from build123d import *

# Parameters (mm, degrees)
SKETCH_2_R          = 6
CUT_EXTRUDE_1_DEPTH = 8
SKETCH_3_W          = 2.5
SKETCH_3_H          = 3
SKETCH_4_W          = 1.25
SKETCH_4_H          = 32


with BuildPart() as part:
    # 草图1 → 旋转1 (revolve)
    with BuildSketch(Plane.XY, mode=Mode.PRIVATE) as revolve_1_sk:
        Polygon((0, 41), (3, 41), (5, 40.647346039), (5, 33.535898385), (3, 33), (3.3865, 33), (4, 32.3865), (4, 18.6135), (3.3865, 18), (2.45, 18), (2.45, 12), (0, 12), align=None)
    revolve(revolve_1_sk.sketch.rotate(Axis((0, 12, 0), (0, 1, 0)), 180), axis=Axis((0, 12, 0), (0, 1, 0)))

    # 草图2 → 切除-拉伸1 (cut)
    with BuildSketch(Plane(origin=(0, 33, 0), x_dir=(1, 0, 0), z_dir=(0, 1, 0))):
        Circle(SKETCH_2_R)
        Polygon((-3.464101615, 0), (-1.732050808, -3), (1.732050808, -3), (3.464101615, 0), (1.732050808, 3), (-1.732050808, 3), align=None, mode=Mode.SUBTRACT)
    extrude(amount=CUT_EXTRUDE_1_DEPTH, mode=Mode.SUBTRACT)

    # 草图3 → 旋转2 (revolve)
    with BuildSketch(Plane.XY, mode=Mode.PRIVATE) as revolve_2_sk:
        with Locations((1.25, 42.5)):
            Rectangle(SKETCH_3_W, SKETCH_3_H)
    revolve(revolve_2_sk.sketch.rotate(Axis((0, 41, 0), (0, 1, 0)), 270), axis=Axis((0, 41, 0), (0, 1, 0)))

    # 草图4 → 切除-旋转1 (revolve, cut)
    with BuildSketch(Plane.XY, mode=Mode.PRIVATE) as cut_revolve_1_sk:
        with Locations((0.625, 28)):
            Rectangle(SKETCH_4_W, SKETCH_4_H)
    revolve(cut_revolve_1_sk.sketch.rotate(Axis((0, 12, 0), (0, 1, 0)), 270), axis=Axis((0, 12, 0), (0, 1, 0)), mode=Mode.SUBTRACT)


solid = part.part
Geometry: final body of the model. Coordinates: model frame, mm. A direction names the side the tool comes from. Round coordinates to 2 decimals unless told otherwise and drop trailing zeros. Loops run counter-clockwise (first coordinate to the right, second up) from the corner with the lowest first, then second, coordinate; pieces in that order, holes last. Notation, with made-up numbers: (21.5, 0.5) - (26.5, 0.5) arc R17 ccw to (26.5, 25.5) - close; hole circle Ø7 at (-7, 22.25). An arc over 180 degrees is marked (long way). Write each question's results on one line, items separated by ' | '. Start each with the question number.
1) Access query for faces 1 (the face through (2.6, 36.9, 1.5)), 2 (the face through (0, 37, -3)), 3 (the face through (2.6, 36.9, -1.5)), 4 (the face through (-2, 41, 2)). Directions: +Z, -Z, +X, -X, +Y, -Y. A direction counts if a zero-diameter tool reaches every point of the face in a straight line with its end or side. Return the directions, or none.
2) Line query: probe 1 along Y at (x, z) = (0.5, -2.5); probe 2 along X at (y, z) = (21.5, 1); probe 3 along Z at (x, y) = (0.75, 39.5). Output: solid intervals per line, ascending. Write a range as [from, to].
3) Cut plane A-A on y = 38.5. Return loops of the section in (x, z), then the cut area to 3 significant figures.
4) Cut plane B-B on y = 15.5. Return loops of the section in (x, z), then the cut area to 3 significant figures.
5) First-contact query: P1, Ø1.5, axis at x = 0, z = 0, coming from the +Y side; P2, Ø1.5, axis at x = 2, z = -2, coming from the -Y side; P3, Ø1.7, axis at x = 1, y = 35.5, coming from the +Z side; P4, Ø4, axis at x = 0.5, y = 36, coming from the -Z side. Flat tips, straight axial feed; report the tip coordinate or a pass-through.
Verdict:
1) face 1: +Z, +X, +Y | face 2: -Z, +X, -X, +Y | face 3: -Z, +X, +Y | face 4: +Y
2) probe 1: y = [18, 41] | probe 2: x = [-3.87, -0.75], [0.75, 3.87] | probe 3: z = [-3, -1], [1, 3]
3) outline: (-3.46, 0) - (-1.73, -3) - (1.73, -3) - (3.46, 0) - (1.73, 3) - (-1.73, 3) - close; hole circle Ø2.5 at (0, 0) | area: 26.3 mm2
4) outline: circle Ø4.9 at (0, 0); hole circle Ø2.5 at (0, 0) | area: 13.9 mm2
5) P1: passes through | P2: stops at y = 12 | P3: stops at z = 3 | P4: stops at z = -3
